Here's how the part is built. I have some questions about the finished solid (model axes, mm). A direction names the side the tool comes from. Coordinates: 2 decimals unless noted, no trailing zeros. Loops run counter-clockwise (first coordinate to the right, second up) from the corner with the lowest first, then second, coordinate; pieces in that order, holes last. Notation, with made-up numbers: (59, -11.75) -> (105, -11.75) arc R18 ccw to (105, 19.25) -> close; hole circle Ø9 at (-32.75, 59.25). An arc over 180 degrees is marked (long way). Answer as a JSON object with one key per item and string values. Group by question number.
1) Which directions (+Z, -Z, +X, -X, +Y, -Y) give clear straight access to the entire face, cutting with the end or side of a thin tool? Please do faces 4 (the flat face through (-6, -53, -29.5)), 5 (the flat face through (-1, -52, 0)).
2) I want a section at A-A (x = -52). Write out the boundary of the cut face in (y, z).
3) I'm going to push a flat-ended pin straight in: pin 1 (9 mm diameter, centred on x = 45, z = -8, fed in from +Y). Where does the tip first touch, or does it pass through?
4) I want a section at B-B (y = 6.5). Write out the boundary of the cut face in (x, z).
5) If we mould it in two halves opening along X, with no side actions, what happens to faces 1 (the flat face through (-1, 52, 0)), 2 (the flat face through (70, -1, 0)), 3 (the flat face through (-6, -53, 29.5))? For each: +X half, -X half, draft (parallel to the pull), parting line (faces both ways), or undercut.
6) I want a section at C-C (z = -8). Write out the boundary of the cut face in (x, y), then the cut area to 3 significant figures.
7) I need wall thicknesses on probe 1 along X at (y, z) = (47, -21.5); probe 2 along Z at (x, y) = (45, 54); probe 3 along Y at (x, z) = (-33, -20). Which ranges of each line are inside material? Lowest first, please. Write a range as [from, to].
8) I want a section at D-D (x = 45). Write out the boundary of the cut face in (y, z), then the cut area to 3 significant figures.
```python
from build123d import *

# Parameters (mm, degrees)
SKETCH_1_W          = 140
SKETCH_1_H          = 110
SKETCH_1_W_2        = 134
SKETCH_1_H_2        = 104
EXTRUDE_1_DEPTH     = 29.5
SKETCH_2_R          = 5.1
CUT_EXTRUDE_1_DEPTH = 70


with BuildPart() as part:
    # 草图1 → 凸台-拉伸1 (new, symmetric)
    with BuildSketch(Plane.XY):
        Rectangle(SKETCH_1_W, SKETCH_1_H)
        Rectangle(SKETCH_1_W_2, SKETCH_1_H_2, mode=Mode.SUBTRACT)
    extrude(amount=EXTRUDE_1_DEPTH, both=True)

    # 草图2 → 切除-拉伸1 (cut, symmetric)
    with BuildSketch(Plane(origin=(0, 0, 0), x_dir=(1, 0, 0), z_dir=(0, 1, 0))):
        with Locations(Location((45, 8, 0), (0, 0, 90))):
            Circle(SKETCH_2_R)
    extrude(amount=CUT_EXTRUDE_1_DEPTH, both=True, mode=Mode.SUBTRACT)


solid = part.part
```
Determined:
{
 "1": {"face 4": "-Z, +X, -X, +Y, -Y", "face 5": "+Z, -Z"},
 "2": {"outline": "(-55, -29.5) -> (-52, -29.5) -> (-52, 29.5) -> (-55, 29.5) -> close; (52, -29.5) -> (55, -29.5) -> (55, 29.5) -> (52, 29.5) -> close"},
 "3": {"pin 1": "through"},
 "4": {"outline": "(-70, -29.5) -> (-67, -29.5) -> (-67, 29.5) -> (-70, 29.5) -> close; (67, -29.5) -> (70, -29.5) -> (70, 29.5) -> (67, 29.5) -> close"},
 "5": {"face 1": "undercut", "face 2": "+X half", "face 3": "draft"},
 "6": {"outline": "(-70, -55) -> (39.9, -55) -> (39.9, -52) -> (-67, -52) -> (-67, 52) -> (39.9, 52) -> (39.9, 55) -> (-70, 55) -> close; (50.1, -55) -> (70, -55) -> (70, 55) -> (50.1, 55) -> (50.1, 52) -> (67, 52) -> (67, -52) -> (50.1, -52) -> close", "area": "1,400 mm^2"},
 "7": {"probe 1": "[-70, -67], [67, 70]", "probe 2": "[-29.5, -13.1], [-2.9, 29.5]", "probe 3": "[-55, -52], [52, 55]"},
 "8": {"outline": "(-55, -29.5) -> (-52, -29.5) -> (-52, -13.1) -> (-55, -13.1) -> close; (-55, -2.9) -> (-52, -2.9) -> (-52, 29.5) -> (-55, 29.5) -> close; (52, -29.5) -> (55, -29.5) -> (55, -13.1) -> (52, -13.1) -> close; (52, -2.9) -> (55, -2.9) -> (55, 29.5) -> (52, 29.5) -> close", "area": "293 mm^2"}
}
